from build123d import *

# Parameters (mm, degrees)
SKETCH1_W                                            = 75
SKETCH1_H                                            = 32
EXTRUDE1_DEPTH                                       = 10
SKETCH2_W                                            = 38.9
SKETCH2_H                                            = 27
EXTRUDE2_DEPTH                                       = 2
CBORE_FOR_M4_HEXAGON_SOCKET_HEAD_CAP_SCR_D           = 4.5
CBORE_FOR_M4_HEXAGON_SOCKET_HEAD_CAP_SCR_CBORE_D     = 8
CBORE_FOR_M4_HEXAGON_SOCKET_HEAD_CAP_SCR_CBORE_DEPTH = 4.6
CBORE_FOR_M5_HEXAGON_SOCKET_HEAD_CAP_SCR_D           = 5.2
CBORE_FOR_M5_HEXAGON_SOCKET_HEAD_CAP_SCR_CBORE_D     = 10
CBORE_FOR_M5_HEXAGON_SOCKET_HEAD_CAP_SCR_CBORE_DEPTH = 5.5
EXTRUDE4_START                                       = 10
EXTRUDE4_DEPTH                                       = 10
SKETCH11_R                                           = 2.5
EXTRUDE6_DEPTH                                       = 2
CHAMFER1_SIZE                                        = 0.5


with BuildPart() as part:
    # Sketch1 → Extrude1 (new body)
    with BuildSketch(Plane(origin=(0, 0, 0), x_dir=(1, 0, 0), z_dir=(0, 1, 0))):
        Rectangle(SKETCH1_W, SKETCH1_H)
    extrude(amount=EXTRUDE1_DEPTH)

    # Sketch2 → Extrude2 (cut)
    with BuildSketch(Plane(origin=(0, 10, 0), x_dir=(1, 0, 0), z_dir=(0, 1, 0))):
        with Locations((18.05, 0)):
            Rectangle(SKETCH2_W, SKETCH2_H)
    extrude(amount=-EXTRUDE2_DEPTH, mode=Mode.SUBTRACT)

    # CBORE for M4 Hexagon socket head cap screws1 (through all)
    with Locations(Plane(origin=(0, 0, 0), x_dir=(-1, 0, 0), z_dir=(0, -1, 0))):
        with Locations((-31.3, -10), (-31.3, 10), (-5.3, 10), (-5.3, -10)):
            CounterBoreHole(CBORE_FOR_M4_HEXAGON_SOCKET_HEAD_CAP_SCR_D / 2, CBORE_FOR_M4_HEXAGON_SOCKET_HEAD_CAP_SCR_CBORE_D / 2, CBORE_FOR_M4_HEXAGON_SOCKET_HEAD_CAP_SCR_CBORE_DEPTH)

    # CBORE for M5 Hexagon socket head cap screws1 (through all)
    with Locations(Plane(origin=(0, 10, 0), x_dir=(1, 0, 0), z_dir=(0, 1, 0))):
        with Locations((-29.5, 10), (-20.5, 10), (-20.5, -10), (-29.5, -10)):
            CounterBoreHole(CBORE_FOR_M5_HEXAGON_SOCKET_HEAD_CAP_SCR_D / 2, CBORE_FOR_M5_HEXAGON_SOCKET_HEAD_CAP_SCR_CBORE_D / 2, CBORE_FOR_M5_HEXAGON_SOCKET_HEAD_CAP_SCR_CBORE_DEPTH)

    # Sketch10 → Extrude4 (cut)
    with BuildSketch(Plane(origin=(0, 4.5, 0), x_dir=(1, 0, 0), z_dir=(0, 1, 0)).offset(EXTRUDE4_START)):
        with BuildLine():
            Line((-29.5, 15), (-20.5, 15))
            ThreePointArc((-20.5, 15), (-15.5, 10), (-20.5, 5))
            Line((-20.5, 5), (-29.5, 5))
            ThreePointArc((-29.5, 5), (-34.5, 10), (-29.5, 15))
        make_face()
        with BuildLine():
            Line((-29.5, -5), (-20.5, -5))
            ThreePointArc((-20.5, -5), (-15.5, -10), (-20.5, -15))
            Line((-20.5, -15), (-29.5, -15))
            ThreePointArc((-29.5, -15), (-34.5, -10), (-29.5, -5))
        make_face()
    extrude(amount=-EXTRUDE4_DEPTH, mode=Mode.SUBTRACT)

    # Sketch11 → Extrude6 (cut)
    with BuildSketch(Plane(origin=(0, 10, 0), x_dir=(1, 0, 0), z_dir=(0, 1, 0))):
        with Locations((-1.4, 11)):
            Circle(SKETCH11_R)
        with Locations((-1.4, -11)):
            Circle(SKETCH11_R)
    extrude(amount=-EXTRUDE6_DEPTH, mode=Mode.SUBTRACT)

    # Chamfer1
    chamfer1_edges = [part.edges().sort_by_distance(p)[0] for p in [
        (0, 10, -16),
        (-37.5, 10, 0),
        (0, 0, -16),
        (0, 0, 16),
        (0, 10, 16),
        (-37.5, 5, -16),
        (37.5, 5, -16),
        (37.5, 5, 16),
        (-37.5, 5, 16),
    ]]
    chamfer(chamfer1_edges, length=CHAMFER1_SIZE)


solid = part.part
For this review, take the finished solid that the model builds, in its own axes (mm). A direction names the side the tool comes from. Coordinates: 2 decimals unless noted, no trailing zeros. Loops run counter-clockwise (first coordinate to the right, second up) from the corner with the lowest first, then second, coordinate; pieces in that order, holes last. Notation, with made-up numbers: (4, -7.75) - (12, -7.75) arc R24 cw to (12, 2.25) - close; hole circle Ø10 at (-35.5, -4). An arc over 180 degrees is marked (long way). Return JSON: item names as keys, results as strings.
Item 1: Take a section at D-D (x = 13.5). Give the boundary of the cut face in (y, z), then the cut area to 4 significant figures.
Determined:
{"outline": "(0, -15.5) - (0.5, -16) - (9.5, -16) - (10, -15.5) - (10, -13.5) - (8, -13.5) - (8, 13.5) - (10, 13.5) - (10, 15.5) - (9.5, 16) - (0.5, 16) - (0, 15.5) - close", "area": "265.5 mm2"}
Item 2: For line 1 (Z direction, x = 5.3, y = 1.7); line 2 (Z direction, x = 5.3, y = 5.95); line 3 (X direction, y = 7, z = 10), list the stretches that pass through material, from the lowest coordinate up.
Determined:
{"line 1": "z = -16 to -14, -6 to 6, 14 to 16", "line 2": "z = -16 to -12.25, -7.75 to 7.75, 12.25 to 16", "line 3": "x = -37.5 to -34.5, -15.5 to 3.05, 7.55 to 29.05, 33.55 to 37.5"}
Item 3: Mouldability with a two-part tool opening along X and no side actions: class faces 1 (the flat face through (-25, 7, 15)), 2 (the flat face through (-1.4, 9, 0)), 3 (the flat face through (-1, 5, -16)) as pulls with the +X half, pulls with the -X half, needs draft (parallel to the pull), parting line crosses it, or undercut.
Determined:
{"face 1": "undercut", "face 2": "pulls with the +X half", "face 3": "needs draft"}
Item 4: Take a section at A-A (x = 5.3). Give the boundary of the cut face in (y, z).
Determined:
{"outline": "(0, -15.5) - (0.5, -16) - (9.5, -16) - (10, -15.5) - (10, -13.5) - (8, -13.5) - (8, -12.25) - (4.6, -12.25) - (4.6, -14) - (0, -14) - close; (0, -6) - (4.6, -6) - (4.6, -7.75) - (8, -7.75) - (8, 7.75) - (4.6, 7.75) - (4.6, 6) - (0, 6) - close; (0, 14) - (4.6, 14) - (4.6, 12.25) - (8, 12.25) - (8, 13.5) - (10, 13.5) - (10, 15.5) - (9.5, 16) - (0.5, 16) - (0, 15.5) - close"}
Item 5: Take a section at C-C (y = 1.25). State how many separate pieces and enclosed holes the cut face has, then the cut area to 3 significant figures.
Determined:
{"separate pieces": "1", "enclosed holes": "8", "area": "2,110 mm2"}
Item 6: For faces 4 (the flat face through (3.6, 4.6, -8.3)), 5 (the flat face through (18, 9, -13.5)), 6 (the flat face through (-25, 4.5, -10)), 7 (the cylindrical face through (5.01, 6.32, 7.77)), list the 3-axis set-ups (+Z, -Z, +X, -X, +Y, -Y) from which the entire face can be reached by the end or side of a thin tool; tool diameter is ignored.
Determined:
{"face 4": "-Y", "face 5": "+X, +Y", "face 6": "+Y", "face 7": "+Y, -Y"}
Item 7: Insertion check: pin 1 (5 mm diameter, centred on x = 5.3, z = -10, fed in from -Y); pin 2 (2.5 mm diameter, centred on x = 5.3, z = 10, fed in from +Y); pin 3 (6 mm diameter, centred on x = -29.5, z = -10, fed in from +Y). Each pin has a flat end and moves straight along its axis. Give the tip position at first contact, or say it passes through.
Determined:
{"pin 1": "stops at y = 4.6", "pin 2": "passes through", "pin 3": "stops at y = 4.5"}
Item 8: Take a section at B-B (z = 0). Give the boundary of the cut face in (x, y), then the cut area to 3 significant figures.
Determined:
{"outline": "(-37.5, 0) - (37.5, 0) - (37.5, 8) - (-1.4, 8) - (-1.4, 10) - (-37, 10) - (-37.5, 9.5) - close", "area": "672 mm2"}
